Can you work these out from the model? Positions are in its coordinate system, mm. Round coordinates to 2 decimals unless told otherwise and drop trailing zeros. Write each loop counter-clockwise with the first axis right and the second up, starting at its lowest first coordinate (ties: lowest second). Pieces come first, ordered by that corner, then holes. Notation, with made-up numbers: (78, -37.75) - (97, -37.75) arc R17 ccw to (97, -18.75) - close; hole circle Ø4 at (-3.5, -39.75). An arc over 180 degrees is marked (long way). One line per item, written item: value. Start each with the question number.
(1) I want a section at A-A on z = 7.25. List the corners of the cut face in (x, y) for me, plus the area to 3 significant figures.
(2) I want a section at B-B on y = 36. List the corners of the cut face in (x, z) for me, plus the area to 3 significant figures.
(3) I want a section at C-C on x = -50. List the corners of the cut face in (y, z) for me.
(4) I'm going to push a flat-ended pin straight in: pin 1 Ø1.5 at (y, z) = (9.5, 10) entering from -X. Where does the tip first touch, or does it pass through?
(5) If I drill on L1, parallel to X at y = 33.5, z = 14.25; L2, parallel to X at y = -23.5, z = 5.25; L3, parallel to Y at x = -32, z = 9, over which ranges is the centre line in solid material (lowest first)? Write a range as from..to.
from build123d import *

# Parameters (mm, degrees)
SKETCH_1_W      = 125
SKETCH_1_H      = 100
EXTRUDE_1_DEPTH = 15
CHAMFER_1_SIZE  = 80


with BuildPart() as part:
    # 草图1 → 凸台-拉伸1 (new body)
    with BuildSketch(Plane.XY):
        Rectangle(SKETCH_1_W, SKETCH_1_H)
    extrude(amount=EXTRUDE_1_DEPTH)

    # 倒角1
    chamfer_1_edges = [part.edges().sort_by_distance(p)[0] for p in [
        (-62.5, 50, 7.5),
    ]]
    chamfer(chamfer_1_edges, length=CHAMFER_1_SIZE)


solid = part.part
Established:
1. outline: (-62.5, -50) - (62.5, -50) - (62.5, 50) - (17.5, 50) - (-62.5, -30) - close
1. area: 9,300 mm2
2. outline: (3.5, 0) - (62.5, 0) - (62.5, 15) - (3.5, 15) - close
2. area: 885 mm2
3. outline: (-50, 0) - (-17.5, 0) - (-17.5, 15) - (-50, 15) - close
4. pin 1: x = -23.75
5. L1: 1..62.5
5. L2: -56..62.5
5. L3: -50..0.5
